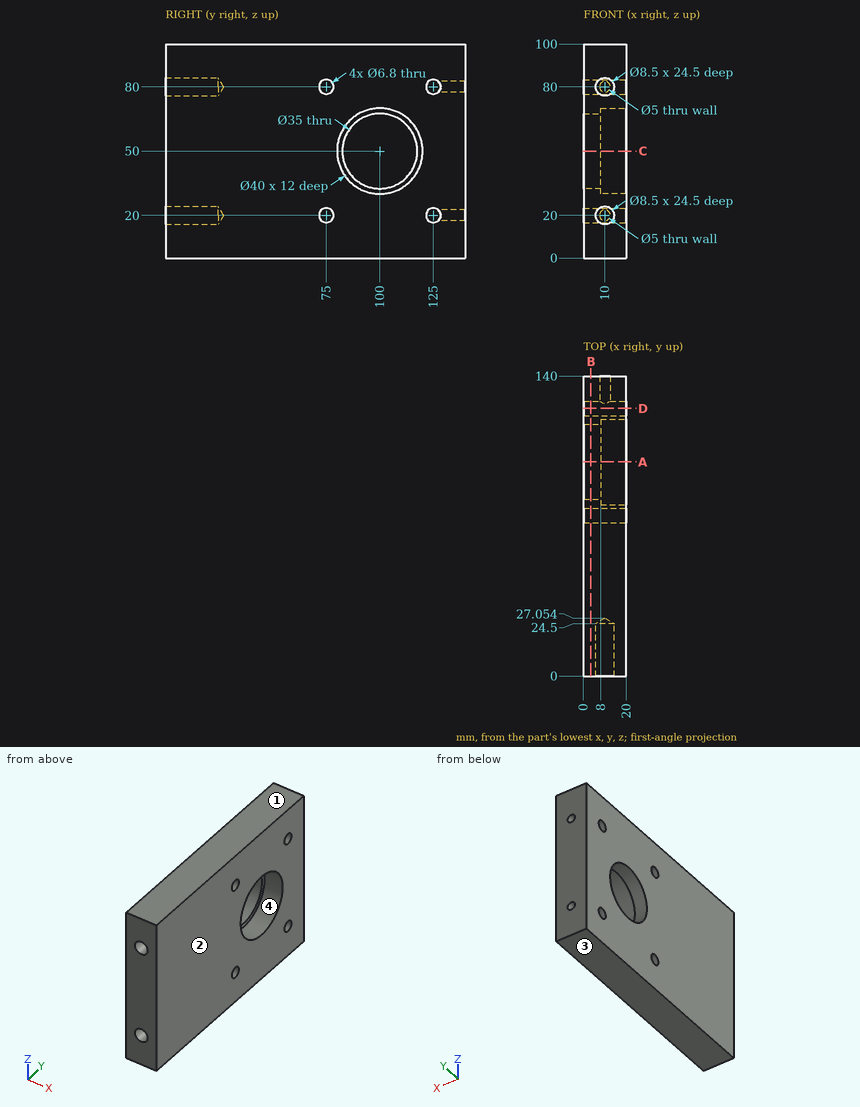
Here's the drawing with two shaded views (mm, measured from the low corner). I have some questions. Give positions to 0.01 mm unless a question says otherwise; leave off trailing zeros. Order: outer loops, then holes, each group sorted by start corner. A loop starts at its lowest first (then second) coordinate and runs counter-clockwise, first axis right, second up. Notation, with made-up numbers: (2, -27.75) - (53, -27.75) arc R22 ccw to (53, -17.75) - close; hole circle Ø1 at (71.5, -15). An arc over 180 degrees is marked (long way). Use a Markdown table: item, result. Add a question column.
Q1. If we section it at A-A on y = 100: Write out the boundary of the cut face in (x, z).
Q2. I'm going to push flat-ended pins straight in: pin 1 (7 mm diameter, centred on x = 10, z = 80, fed in from +Y); pin 2 (8 mm diameter, centred on x = 10, z = 80, fed in from -Y); pin 3 (3 mm diameter, centred on x = 10, z = 20, fed in from +Y). Where does each tip first touch, or does it pass through?
Q3. Please list where these lines run through material, in increasing order: line 1 along Z through (x, y) = (10, 12); line 2 along Y through (x, z) = (5.5, 20); line 3 along X through (y, z) = (133.25, 20).
Q4. If we section it at D-D on y = 125: Write out the boundary of the cut face in (x, z).
Q5. If we section it at B-B on x = 3.5: Write out the boundary of the cut face in (y, z), plus the area to 3 significant figures.
Q6. If we mould it in two halves opening along Z, with no side actions, what happens to the marked faces 1, 2, 3 and 4? For each: released by +Z, released by -Z, zero draft, split by the parting line, or undercut.
Q7. If we section it at C-C on z = 50: Write out the boundary of the cut face in (x, y).
Answers follow:
| question | item | result |
|---|---|---|
| 1 | outline | (0, 0) - (20, 0) - (20, 30) - (8, 30) - (8, 32.5) - (0, 32.5) - close; (0, 67.5) - (8, 67.5) - (8, 70) - (20, 70) - (20, 100) - (0, 100) - close |
| 2 | pin 1 | stops at y = 140 |
| 2 | pin 2 | stops at y = 24.65 |
| 2 | pin 3 | stops at y = 121.95 |
| 3 | line 1 | z = 0 to 15.75, 24.25 to 75.75, 84.25 to 100 |
| 3 | line 2 | y = 0 to 71.6, 78.4 to 121.6, 128.4 to 140 |
| 3 | line 3 | x = 0 to 7.5, 12.5 to 20 |
| 4 | outline | (0, 0) - (20, 0) - (20, 16.6) - (0, 16.6) - close; (0, 23.4) - (20, 23.4) - (20, 76.6) - (0, 76.6) - close; (0, 83.4) - (20, 83.4) - (20, 100) - (0, 100) - close |
| 5 | outline | (0, 0) - (140, 0) - (140, 100) - (0, 100) - close; hole circle Ø6.8 at (75, 20); hole circle Ø6.8 at (75, 80); hole circle Ø35 at (100, 50); hole circle Ø6.8 at (125, 20); hole circle Ø6.8 at (125, 80) |
| 5 | area | 12,900 mm^2 |
| 6 | face 1 | released by +Z |
| 6 | face 2 | zero draft |
| 6 | face 3 | released by -Z |
| 6 | face 4 | undercut |
| 7 | outline | (0, 0) - (20, 0) - (20, 80) - (8, 80) - (8, 82.5) - (0, 82.5) - close; (0, 117.5) - (8, 117.5) - (8, 120) - (20, 120) - (20, 140) - (0, 140) - close |
